from build123d import *

# Parameters (mm, degrees)
SKETCH1_R                                         = 55
SKETCH1_R_2                                       = 25
BOSS_EXTRUDE1_DEPTH                               = 20
CUT_EXTRUDE1_DEPTH                                = 10
CHAMFER1_SIZE                                     = 5
CSK_FOR_8_FLAT_HEAD_MACHINE_SCREW_100_D           = 4.9149
CSK_FOR_8_FLAT_HEAD_MACHINE_SCREW_100_CSINK_D     = 8.4328
CSK_FOR_8_FLAT_HEAD_MACHINE_SCREW_100_CSINK_ANGLE = 100
MIRROR2_COPY_1_D                                  = 4.9149
MIRROR2_COPY_1_CSINK_D                            = 8.4328
MIRROR2_COPY_1_CSINK_ANGLE                        = 100


with BuildPart() as part:
    # Sketch1 → Boss-Extrude1 (new body)
    with BuildSketch(Plane.XY):
        Circle(SKETCH1_R)
        Circle(SKETCH1_R_2, mode=Mode.SUBTRACT)
    extrude(amount=BOSS_EXTRUDE1_DEPTH)

    # Sketch2 → Cut-Extrude1 (cut)
    with BuildSketch(Plane.XY.offset(20)):
        with BuildLine():
            Line((-10.612144625, 28.060334753), (-19.017070243, 40.784200855))
            ThreePointArc((-19.017070243, 40.784200855), (-33.794395167, 29.714287056), (-42.88237403, 13.641920597))
            Line((-42.88237403, 13.641920597), (-28.060334753, 10.612144625))
            ThreePointArc((-28.060334753, 10.612144625), (-21.213203436, 21.213203436), (-10.612144625, 28.060334753))
        make_face()
        with BuildLine():
            Line((28.060334753, 10.612144625), (42.88237403, 13.641920597))
            ThreePointArc((42.88237403, 13.641920597), (33.794395167, 29.714287056), (19.017070243, 40.784200855))
            Line((19.017070243, 40.784200855), (10.612144625, 28.060334753))
            ThreePointArc((10.612144625, 28.060334753), (21.213203436, 21.213203436), (28.060334753, 10.612144625))
        make_face()
        with BuildLine():
            Line((10.612144625, -28.060334753), (19.017070243, -40.784200855))
            ThreePointArc((19.017070243, -40.784200855), (33.794395167, -29.714287056), (42.88237403, -13.641920597))
            Line((42.88237403, -13.641920597), (28.060334753, -10.612144625))
            ThreePointArc((28.060334753, -10.612144625), (21.213203436, -21.213203436), (10.612144625, -28.060334753))
        make_face()
        with BuildLine():
            Line((-28.060334753, -10.612144625), (-42.88237403, -13.641920597))
            ThreePointArc((-42.88237403, -13.641920597), (-33.794395167, -29.714287056), (-19.017070243, -40.784200855))
            Line((-19.017070243, -40.784200855), (-10.612144625, -28.060334753))
            ThreePointArc((-10.612144625, -28.060334753), (-21.213203436, -21.213203436), (-28.060334753, -10.612144625))
        make_face()
    extrude(amount=-CUT_EXTRUDE1_DEPTH, mode=Mode.SUBTRACT)

    # Chamfer1
    chamfer1_edges = [part.edges().sort_by_distance(p)[0] for p in [
        (-55, 0, 20),
    ]]
    chamfer(chamfer1_edges, length=CHAMFER1_SIZE)

    # CSK for #8 Flat Head Machine Screw (100)1 (through all)
    with Locations(Plane(origin=(-28.284271247, 26.457513111, 10), x_dir=(1, 0, 0), z_dir=(0, 0, 1))):
        with Locations((0, 0)):
            csk_for_8_flat_head_machine_screw_100 = CounterSinkHole(CSK_FOR_8_FLAT_HEAD_MACHINE_SCREW_100_D / 2, CSK_FOR_8_FLAT_HEAD_MACHINE_SCREW_100_CSINK_D / 2, counter_sink_angle=CSK_FOR_8_FLAT_HEAD_MACHINE_SCREW_100_CSINK_ANGLE)

    # Mirror1: CSK for #8 Flat Head Machine Screw (100)1 across plane
    add(csk_for_8_flat_head_machine_screw_100.mirror(Plane(origin=(0, 0, 0), x_dir=(0, 0, 1), z_dir=(1, 0, 0))), mode=Mode.SUBTRACT)

    # Mirror2: CSK for #8 Flat Head Machine Screw (100)1 across plane
    add(csk_for_8_flat_head_machine_screw_100.mirror(Plane.ZX), mode=Mode.SUBTRACT)

    # Mirror2 copy 1 (through all)
    with Locations(Plane(origin=(28.284271247, -26.457513111, 10), x_dir=(-1, 0, 0), z_dir=(0, 0, 1))):
        with Locations((0, 0)):
            CounterSinkHole(MIRROR2_COPY_1_D / 2, MIRROR2_COPY_1_CSINK_D / 2, counter_sink_angle=MIRROR2_COPY_1_CSINK_ANGLE)


solid = part.part
The model under review builds one solid part; all positions refer to its coordinate system, in mm. A direction names the side the tool comes from. Coordinates: 2 decimals unless noted, no trailing zeros. Loops run counter-clockwise (first coordinate to the right, second up) from the corner with the lowest first, then second, coordinate; pieces in that order, holes last. Notation, with made-up numbers: (35, -4) -> (40, -4) arc R9 cw to (40, 10) -> close; hole circle Ø7 at (33.5, 87). An arc over 180 degrees is marked (long way). Use a Markdown table: item, result. Add a question column.
1. To check wall thickness, follow line 1 (Y direction, x = -41, z = 17); line 2 (X direction, y = 27, z = 10.75); line 3 (X direction, y = -23, z = 16). State the ranges of each line that lie inside material, in increasing order.
2. Machinability: for faces 1 (the face through (-14.756, 34.333, 15.07)), 2 (the face through (-26.473, -28.118, 4.202)), which of the approach directions +Z, -Z, +X, -X, +Y, -Y give a long, thin tool a straight path to every point of the face, cutting with its end or side? Answer none if there is none.
3. Add section C-C on z = 17. Write out the cut boundary in (x, y), plus the area to 3 significant figures.
4. Add section A-A on y = 0. Write out the cut boundary in (x, z).
5. Add section D-D on z = 5.5. Write out the cut boundary in (x, y).
6. Clearance check with flat-ended pins moving along their axes: pin 1 Ø8 at (x, y) = (-21.5, 34) entering from -Z; pin 2 Ø4 at (y, z) = (-32, 12.5) entering from +X; pin 3 Ø1 at (y, z) = (-8, 6.5) entering from -X; pin 4 Ø2 at (x, z) = (4.5, 17) entering from +Y. State where each tip first meets the part, or that it passes through.
7. Draft analysis for pull direction Y (two halves, no side actions). For faces 3 (the face through (-11.923, -53.692, 7.395)), 4 (the face through (23.846, 7.509, 9.86)), state which applies: pulls with the +Y half, pulls with the -Y half, needs draft (parallel to the pull), parting line crosses it, or undercut.
Returned:
| question | item | result |
|---|---|---|
| 1 | line 1 | y = -33.59 to -18.55, -13.26 to 13.26, 18.55 to 33.59 |
| 1 | line 2 | x = -47.92 to -36, -13.08 to 13.08, 36 to 47.92 |
| 1 | line 3 | x = -48.86 to -38.68, -19.26 to -9.8, 9.8 to 19.26, 38.68 to 48.86 |
| 2 | face 1 | +Z |
| 2 | face 2 | +Z, -Z |
| 3 | outline | circle Ø106 at (0, 0); hole (-42.88, -13.64) arc R45 ccw to (-19.02, -40.78) -> (-10.61, -28.06) arc R30 cw to (-28.06, -10.61) -> close; hole (-42.88, 13.64) -> (-28.06, 10.61) arc R30 cw to (-10.61, 28.06) -> (-19.02, 40.78) arc R45 ccw to start; hole circle Ø50 at (0, 0); hole (10.61, -28.06) -> (19.02, -40.78) arc R45 ccw to (42.88, -13.64) -> (28.06, -10.61) arc R30 cw to start; hole (10.61, 28.06) arc R30 cw to (28.06, 10.61) -> (42.88, 13.64) arc R45 ccw to (19.02, 40.78) -> close |
| 3 | area | 4,980 mm² |
| 4 | outline | (-55, 0) -> (-25, 0) -> (-25, 20) -> (-50, 20) -> (-55, 15) -> close; (25, 0) -> (55, 0) -> (55, 15) -> (50, 20) -> (25, 20) -> close |
| 5 | outline | circle Ø110 at (0, 0); hole circle Ø4.91 at (-28.28, -26.46); hole circle Ø4.91 at (-28.28, 26.46); hole circle Ø50 at (0, 0); hole circle Ø4.91 at (28.28, -26.46); hole circle Ø4.91 at (28.28, 26.46) |
| 6 | pin 1 | stops at z = 0 |
| 6 | pin 2 | stops at x = 46.1 |
| 6 | pin 3 | stops at x = -54.49 |
| 6 | pin 4 | stops at y = 53.82 |
| 7 | face 3 | parting line crosses it |
| 7 | face 4 | undercut |
